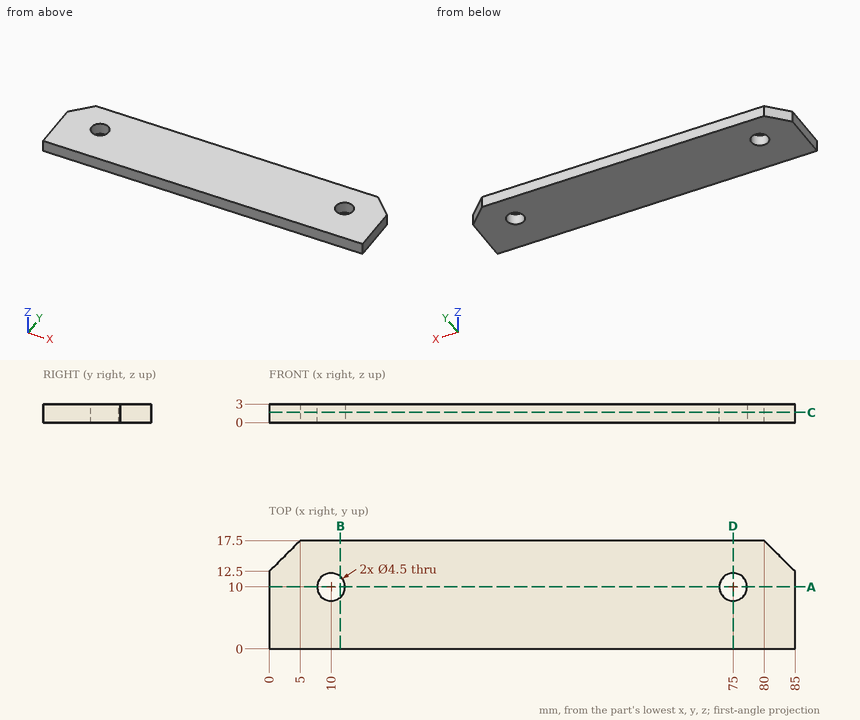
Verification items for this drawing (mm, ordinates from the low corner). Coordinates: 2 decimals unless noted, no trailing zeros. Loops run counter-clockwise (first coordinate to the right, second up) from the corner with the lowest first, then second, coordinate; pieces in that order, holes last. Notation, with made-up numbers: (69, 31) - (106, 31) arc R21 cw to (106, 69) - close; hole circle Ø4 at (-30, 79). An arc over 180 degrees is marked (long way). Use one line per item in the form item = value. Start each with the question number.
Item 1: Section check A-A, the plane y = 10. Enter the section's corners in (x, z).
Item 2: Thickness scan on probe 1 along Y at (x, z) = (10, 1.2); probe 2 along X at (y, z) = (10.75, 2.4); probe 3 along X at (y, z) = (8, 0.75). Record the ranges inside material, lowest first.
Item 3: Section check B-B, the plane x = 11.5. Enter the section's corners in (y, z), and give its area (3 significant figures).
Item 4: Gauge pin test, flat end, axial feed: pin 1 (6 mm diameter, centred on x = 75, y = 10, fed in from -Z). Record the tip position at first contact, or that the pin passes through.
Item 5: Section check C-C, the plane z = 1.65. Enter the section's corners in (x, y).
Item 6: Section check D-D, the plane x = 75. Enter the section's corners in (y, z).
Computed:
q1.outline = (0, 0) - (7.75, 0) - (7.75, 3) - (0, 3) - close; (12.25, 0) - (72.75, 0) - (72.75, 3) - (12.25, 3) - close; (77.25, 0) - (85, 0) - (85, 3) - (77.25, 3) - close
q2.probe_1 = 0 to 7.75, 12.25 to 17.5
q2.probe_2 = 0 to 7.88, 12.12 to 72.88, 77.12 to 85
q2.probe_3 = 0 to 8.97, 11.03 to 73.97, 76.03 to 85
q3.outline = (0, 0) - (8.32, 0) - (8.32, 3) - (0, 3) - close; (11.68, 0) - (17.5, 0) - (17.5, 3) - (11.68, 3) - close
q3.area = 42.4 mm2
q4.pin_1 = 0
q5.outline = (0, 0) - (85, 0) - (85, 12.5) - (80, 17.5) - (5, 17.5) - (0, 12.5) - close; hole circle Ø4.5 at (10, 10); hole circle Ø4.5 at (75, 10)
q6.outline = (0, 0) - (7.75, 0) - (7.75, 3) - (0, 3) - close; (12.25, 0) - (17.5, 0) - (17.5, 3) - (12.25, 3) - close
